```python
from build123d import *

# Parameters (mm, degrees)
BOSS_EXTRUDE1_DEPTH   = 4
M8_TAPPED_HOLE1_D     = 6.8
M8_TAPPED_HOLE1_DEPTH = 22.25
M8_TAPPED_HOLE1_TIP   = 2.042926105
CHAMFER1_SIZE         = 2


with BuildPart() as part:
    # Sketch1 → Boss-Extrude1 (new, symmetric)
    with BuildSketch(Plane(origin=(0, 0, 0), x_dir=(0, 0, -1), z_dir=(1, 0, 0))):
        with BuildLine():
            Line((-9, 0), (9, 0))
            Line((9, 0), (9, 35))
            ThreePointArc((9, 35), (0, 44), (-9, 35))
            Line((-9, 35), (-9, 0))
        make_face()
        with BuildLine():
            Line((3.25, 17), (3.25, 7))
            ThreePointArc((3.25, 7), (0, 3.75), (-3.25, 7))
            Line((-3.25, 7), (-3.25, 17))
            ThreePointArc((-3.25, 17), (0, 20.25), (3.25, 17))
        make_face(mode=Mode.SUBTRACT)
    extrude(amount=BOSS_EXTRUDE1_DEPTH, both=True)

    # M8 Tapped Hole1
    with Locations(Plane.ZY.offset(4)):
        with Locations((0, 35)):
            Hole(M8_TAPPED_HOLE1_D / 2, depth=M8_TAPPED_HOLE1_DEPTH)
            with Locations((0, 0, -(M8_TAPPED_HOLE1_DEPTH + M8_TAPPED_HOLE1_TIP / 2))):  # 118° drill point
                Cone(0, M8_TAPPED_HOLE1_D / 2, M8_TAPPED_HOLE1_TIP, mode=Mode.SUBTRACT)

    # Chamfer1
    chamfer1_edges = [part.edges().sort_by_distance(p)[0] for p in [
        (0, 0, -9),
        (0, 0, 9),
    ]]
    chamfer(chamfer1_edges, length=CHAMFER1_SIZE)


solid = part.part
```
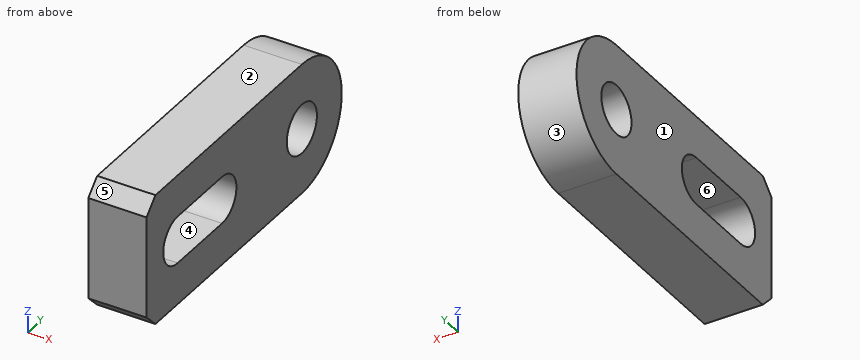
The model under review builds one solid part; all positions refer to its coordinate system, in mm. Face numbers are marked on the shaded views. A direction names the side the tool comes from. Round coordinates to 2 decimals unless told otherwise and drop trailing zeros. Order: outer loops, then holes, each group sorted by start corner. A loop starts at its lowest first (then second) coordinate and runs counter-clockwise, first axis right, second up. Notation, with made-up numbers: (-5.75, -27.75) -> (50.25, -27.75) arc R14 cw to (50.25, -5.75) -> close; hole circle Ø10 at (5, -8). An arc over 180 degrees is marked (long way). One line per item, written item: value. Start each with the question number.
Q1. Take a section at A-A (z = 0). Write out the cut boundary in (x, y), and give its area (3 significant figures).
Q2. Mouldability with a two-part tool opening along Z and no side actions: class the marked faces 1, 2, 3 and 4 as released by +Z, released by -Z, zero draft, split by the parting line, or undercut.
Q3. Take a section at B-B (x = 3.25). Write out the cut boundary in (y, z), and give its area (3 significant figures).
Q4. Machinability: for the marked faces 5 and 6, which of the approach directions +Z, -Z, +X, -X, +Y, -Y give a long, thin tool a straight path to every point of the face, cutting with its end or side? Answer none if there is none.
Q5. Take a section at C-C (y = 38). Write out the cut boundary in (x, z).
Q6. Wall thickness on line 1 (Y direction, x = -2, z = 0); line 2 (Z direction, x = 3.75, y = 12.5); line 3 (Y direction, x = 1, z = -2.5): over which ranges is each line inside the solid? List them lowest first.
Reported:
1. outline: (-4, 0) -> (4, 0) -> (4, 3.75) -> (-4, 3.75) -> close; (-4, 20.25) -> (4, 20.25) -> (4, 31.6) -> (-4, 31.6) -> close; (-4, 38.4) -> (4, 38.4) -> (4, 44) -> (-4, 44) -> close
1. area: 166 mm2
2. face 1: zero draft
2. face 2: released by +Z
2. face 3: split by the parting line
2. face 4: undercut
3. outline: (0, -7) -> (2, -9) -> (35, -9) arc R9 ccw to (35, 9) -> (2, 9) -> (0, 7) -> close; hole (7, -3.25) -> (17, -3.25) arc R3.25 ccw to (17, 3.25) -> (7, 3.25) arc R3.25 ccw to start; hole circle Ø6.8 at (35, 0)
3. area: 619 mm2
4. face 5: +Z, +X, -X, -Y
4. face 6: +X, -X
5. outline: (-4, -8.49) -> (4, -8.49) -> (4, -1.6) -> (-4, -1.6) -> close; (-4, 1.6) -> (4, 1.6) -> (4, 8.49) -> (-4, 8.49) -> close
6. line 1: y = 0 to 3.75, 20.25 to 31.6, 38.4 to 44
6. line 2: z = -9 to -3.25, 3.25 to 9
6. line 3: y = 0 to 4.92, 19.08 to 32.7, 37.3 to 43.65
